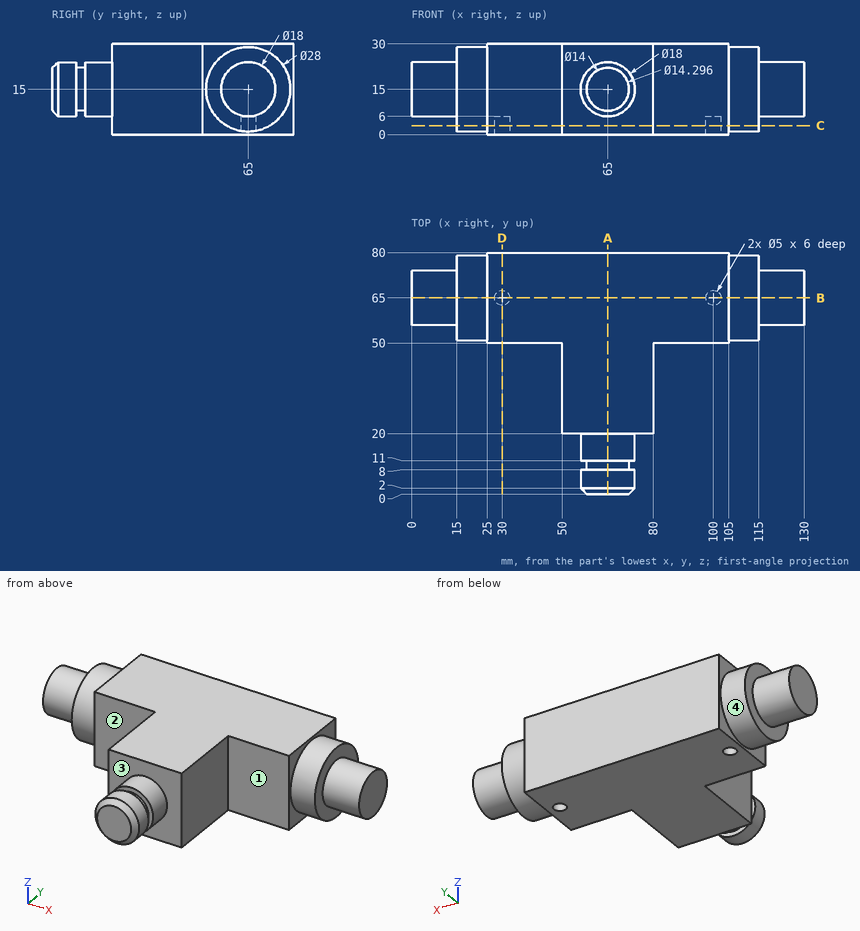
Part print with two shaded views. Sizes in mm from the minimum x, y, z corner. A direction names the side the tool comes from. Coordinates: 2 decimals unless noted, no trailing zeros. Write each loop counter-clockwise with the first axis right and the second up, starting at its lowest first coordinate (ties: lowest second). Pieces come first, ordered by that corner, then holes. Notation, with made-up numbers: (30, 17) - (55, 17) arc R17 ccw to (55, 33) - close; hole circle Ø4 at (7.5, -30.75). An arc over 180 degrees is marked (long way). One line per item, written item: value. Start each with the question number.
1. Slice it at B-B (y = 65). Write the cut outline in (x, z).
2. Slice it at C-C (z = 3). Write the cut outline in (x, y).
3. Probe line 1 (Y direction, x = 100, z = 2.05); line 2 (Y direction, x = 91, z = 11). List the from-to ranges inside material, lowest first. Write a range as from..to.
4. Slice it at A-A (x = 65). Write the cut outline in (y, z).
5. Flat gauge pins, fed straight in: pin 1 (8 mm diameter, centred on y = 16.5, z = 18, fed in from -X); pin 2 (9 mm diameter, centred on y = 29.5, z = 15.5, fed in from +X); pin 3 (7.5 mm diameter, centred on x = 33, z = 21, fed in from -Y). Where does each tip first touch, or does it go through?
6. Tool access for the marked faces 1, 2, 3 and 4: list every direction of +Z, -Z, +X, -X, +Y, -Y with a clear straight run to the whole face (end or side of a thin tool).
7. Slice it at D-D (x = 30). Write the cut outline in (y, z), plus the area to 3 significant figures.
Answers below:
1. outline: (0, 6) - (15, 6) - (15, 1) - (25, 1) - (25, 0) - (27.5, 0) - (27.5, 6) - (32.5, 6) - (32.5, 0) - (97.5, 0) - (97.5, 6) - (102.5, 6) - (102.5, 0) - (105, 0) - (105, 1) - (115, 1) - (115, 6) - (130, 6) - (130, 24) - (115, 24) - (115, 29) - (105, 29) - (105, 30) - (25, 30) - (25, 29) - (15, 29) - (15, 24) - (0, 24) - close
2. outline: (15, 57.79) - (25, 57.79) - (25, 50) - (50, 50) - (50, 20) - (80, 20) - (80, 50) - (105, 50) - (105, 57.79) - (115, 57.79) - (115, 72.21) - (105, 72.21) - (105, 80) - (25, 80) - (25, 72.21) - (15, 72.21) - close; hole circle Ø5 at (30, 65); hole circle Ø5 at (100, 65)
3. line 1: y = 50..62.5, 67.5..80
3. line 2: y = 50..80
4. outline: (0, 8) - (2, 6) - (8, 6) - (8, 7.85) - (11, 7.85) - (11, 6) - (20, 6) - (20, 0) - (80, 0) - (80, 30) - (20, 30) - (20, 24) - (11, 24) - (11, 22.15) - (8, 22.15) - (8, 24) - (2, 24) - (0, 22) - close
5. pin 1: stops at x = 50
5. pin 2: stops at x = 80
5. pin 3: stops at y = 50
6. face 1: +Z, -Z, +X, -Y
6. face 2: +Z, -Z, -X, -Y
6. face 3: -Y
6. face 4: -X
7. outline: (50, 0) - (62.5, 0) - (62.5, 6) - (67.5, 6) - (67.5, 0) - (80, 0) - (80, 30) - (50, 30) - close
7. area: 870 mm^2
